Answer from the drawing. Dimensions are ordinates in mm from the lowest x, y and z of the part. Give positions to 0.01 mm unless a question says otherwise; leave off trailing zeros. Write each loop counter-clockwise with the first axis right and the second up, starting at its lowest first coordinate (ties: lowest second). Pieces come first, ordered by that corner, then holes. Notation, with made-up numbers: (7, 40.25) -> (53, 40.25) arc R24 ccw to (53, 55.25) -> close; hole circle Ø8 at (19.25, 8.25). An arc over 180 degrees is marked (long way). Write item = value, one per line.
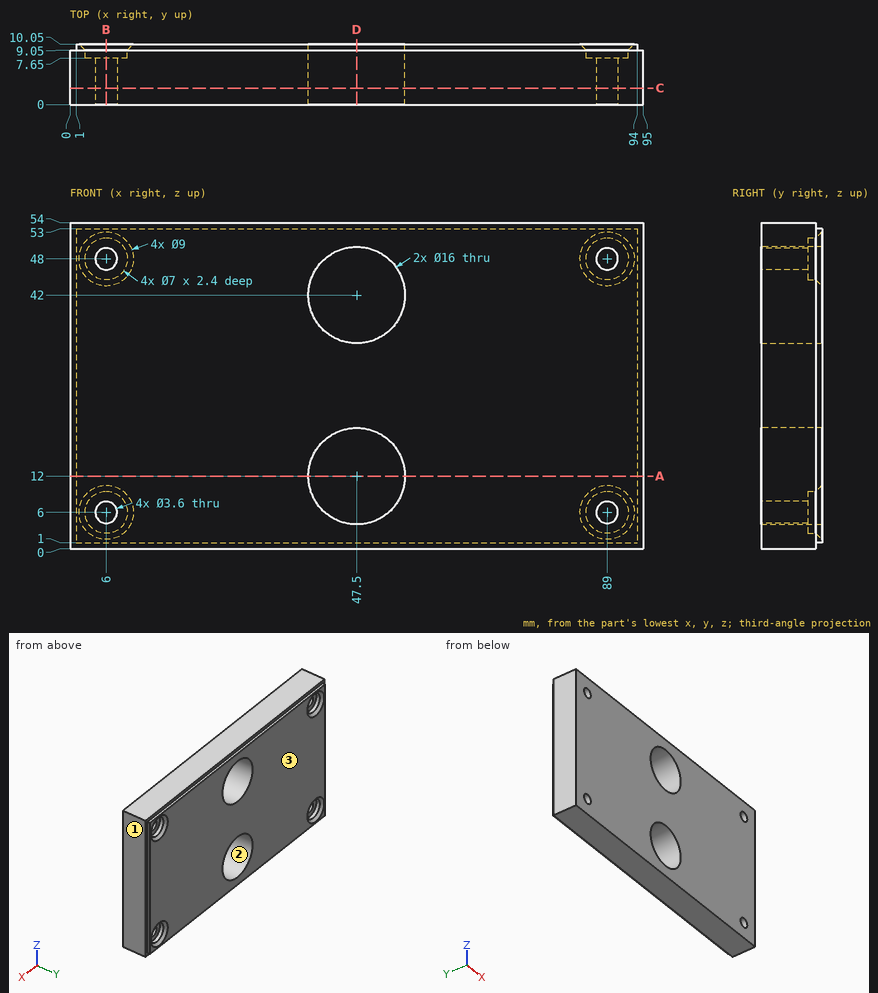
(1) Given P1, Ø7.5, axis at x = 5.5, z = 5.5, coming from the +Y side; P2, Ø1, axis at y = 4.5, z = 37, coming from the -X side; P3, Ø5.5, axis at x = 90, z = 6, coming from the +Y side; P4, Ø4.5, axis at x = 6, z = 6, coming from the +Y side, each flat-ended and moving along its own axis, determine where each tip first touches the part or whether it passes through.
Checks:
P1 = 10.01
P2 = 0
P3 = 9.3
P4 = 7.65
(2) The part is cut by section A-A on z = 12. Determine the outline of the cut face in (x, y), plus the area to 3 significant figures.
Checks:
outline = (0, 0) -> (39.5, 0) -> (39.5, 10.05) -> (1, 10.05) -> (1, 9.05) -> (0, 9.05) -> close; (55.5, 0) -> (95, 0) -> (95, 9.05) -> (94, 9.05) -> (94, 10.05) -> (55.5, 10.05) -> close
area = 792 mm²
(3) The part is cut by section B-B on x = 6. Determine the outline of the cut face in (y, z).
Checks:
outline = (0, 0) -> (9.05, 0) -> (9.05, 1) -> (10.05, 1) -> (10.05, 1.5) -> (9.05, 2.5) -> (7.65, 2.5) -> (7.65, 4.2) -> (0, 4.2) -> close; (0, 7.8) -> (7.65, 7.8) -> (7.65, 9.5) -> (9.05, 9.5) -> (10.05, 10.5) -> (10.05, 43.5) -> (9.05, 44.5) -> (7.65, 44.5) -> (7.65, 46.2) -> (0, 46.2) -> close; (0, 49.8) -> (7.65, 49.8) -> (7.65, 51.5) -> (9.05, 51.5) -> (10.05, 52.5) -> (10.05, 53) -> (9.05, 53) -> (9.05, 54) -> (0, 54) -> close
(4) For a pull along X with two mould halves and no side action, classify the marked faces 1, 2 and 3 as released by +X, released by -X, zero draft, split by the parting line, or undercut.
Checks:
face_1 = released by +X
face_2 = undercut
face_3 = zero draft
(5) The part is cut by section C-C on y = 2.75. Determine the outline of the cut face in (x, z), plus the area to 3 significant figures.
Checks:
outline = (0, 0) -> (95, 0) -> (95, 54) -> (0, 54) -> close; hole circle Ø3.6 at (6, 6); hole circle Ø3.6 at (6, 48); hole circle Ø16 at (47.5, 12); hole circle Ø16 at (47.5, 42); hole circle Ø3.6 at (89, 6); hole circle Ø3.6 at (89, 48)
area = 4,690 mm²
(6) Consider L1, parallel to Z at x = 89, y = 5.5; L2, parallel to X at y = 8.1, z = 6; L3, parallel to X at y = 5.25, z = 7.5. Determine where each line is inside the solid, lowest interval first.
Checks:
L1 = 0 to 4.2, 7.8 to 46.2, 49.8 to 54
L2 = 0 to 2.5, 9.5 to 42.21, 52.79 to 85.5, 92.5 to 95
L3 = 0 to 5.01, 6.99 to 40.89, 54.11 to 88.01, 89.99 to 95
(7) The part is cut by section D-D on x = 47.5. Determine the outline of the cut face in (y, z), plus the area to 3 significant figures.
Checks:
outline = (0, 0) -> (9.05, 0) -> (9.05, 1) -> (10.05, 1) -> (10.05, 4) -> (0, 4) -> close; (0, 20) -> (10.05, 20) -> (10.05, 34) -> (0, 34) -> close; (0, 50) -> (10.05, 50) -> (10.05, 53) -> (9.05, 53) -> (9.05, 54) -> (0, 54) -> close
area = 219 mm²
